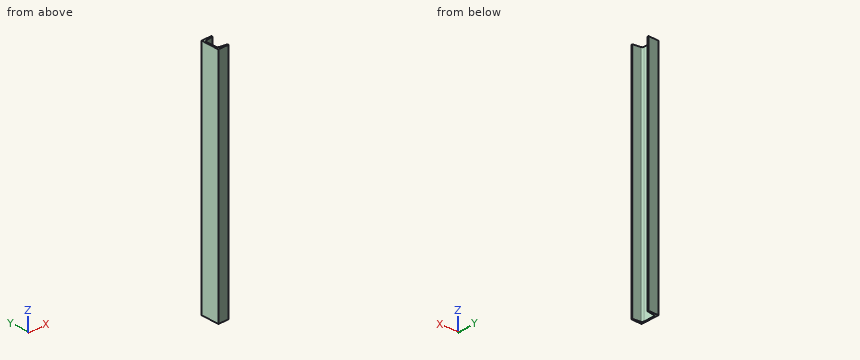
from build123d import *

# Parameters (mm, degrees)
BOSS_EXTRUDE1_DEPTH = 1022


with BuildPart() as part:
    # Sketch1 → Boss-Extrude1 (new body)
    with BuildSketch(Plane.XY):
        with BuildLine():
            Line((0, 0), (-45, 0))
            Line((-45, 0), (-45, -80))
            Line((-45, -80), (0, -80))
            Line((0, -80), (0, -78.639315732))
            ThreePointArc((0, -78.639315732), (-0.981161679, -76.015079616), (-3.443307596, -74.678243457))
            Line((-3.443307596, -74.678243457), (-32.113384808, -70.648926875))
            ThreePointArc((-32.113384808, -70.648926875), (-37.037676642, -67.975254557), (-39, -62.726782325))
            Line((-39, -62.726782325), (-39, -17.273217675))
            ThreePointArc((-39, -17.273217675), (-37.037676642, -12.024745443), (-32.113384808, -9.351073125))
            Line((-32.113384808, -9.351073125), (-3.443307596, -5.321756543))
            ThreePointArc((-3.443307596, -5.321756543), (-0.981161679, -3.984920384), (0, -1.360684268))
            Line((0, -1.360684268), (0, 0))
        make_face()
    extrude(amount=BOSS_EXTRUDE1_DEPTH)


solid = part.part
For this review, take the finished solid that the model builds, in its own axes (mm). Give positions to 0.01 mm unless a question says otherwise; leave off trailing zeros. Write each loop counter-clockwise with the first axis right and the second up, starting at its lowest first coordinate (ties: lowest second). Pieces come first, ordered by that corner, then holes. Notation, with made-up numbers: (28.5, -26) -> (76.5, -26) arc R13 ccw to (76.5, -22) -> close; hole circle Ø7 at (38.5, 15.5). An arc over 180 degrees is marked (long way). Use CSV: the item, a comma, the result in double quotes.
Q1. For P1, Ø1, axis at x = -39.5, y = -58.5, coming from the -Z side; P2, Ø3, axis at y = -24.5, z = 747.5, coming from the +X side; P3, Ø4, axis at y = -17.5, z = 864, coming from the +X side; P4, Ø8, axis at x = -23, y = -64.5, coming from the -Z side, all flat-tipped, find the tip position at first contact; note any pin that passes through.
Conclusion:
P1,"z = 0"
P2,"x = -39"
P3,"x = -38.8"
P4,"through"
Q2. To check wall thickness, follow probe 1 along Y at (x, z) = (-31, 201); probe 2 along Y at (x, z) = (-4.5, 657); probe 3 along X at (y, z) = (-27.5, 650). State the ranges of each line that lie inside material, in increasing order. Write a range as [from, to].
Conclusion:
probe 1,"[-80, -70.81], [-9.19, 0]"
probe 2,"[-80, -74.53], [-5.47, 0]"
probe 3,"[-45, -39]"
Q3. Take a section at A-A, the plane z = 156. Write out the cut boundary in (x, y), then the cut area to 3 significant figures.
Conclusion:
outline,"(-45, -80) -> (0, -80) -> (0, -78.64) arc R4 ccw to (-3.44, -74.68) -> (-32.11, -70.65) arc R8 cw to (-39, -62.73) -> (-39, -17.27) arc R8 cw to (-32.11, -9.35) -> (-3.44, -5.32) arc R4 ccw to (0, -1.36) -> (0, 0) -> (-45, 0) -> close"
area,"1,090 mm2"
Q4. Take a section at C-C, the plane y = -37.5. Write out the cut boundary in (x, z), then the cut area to 3 significant figures.
Conclusion:
outline,"(-45, 0) -> (-39, 0) -> (-39, 1022) -> (-45, 1022) -> close"
area,"6,130 mm2"
Q5. Take a section at B-B, the plane x = -18. Write out the cut boundary in (y, z), then the cut area to 3 significant figures.
Conclusion:
outline,"(-80, 0) -> (-72.63, 0) -> (-72.63, 1022) -> (-80, 1022) -> close; (-7.37, 0) -> (0, 0) -> (0, 1022) -> (-7.37, 1022) -> close"
area,"15,100 mm2"
